from build123d import *

# Parameters (mm, degrees)
BOSS_EXTRUDE1_DEPTH = 20
BOSS_EXTRUDE2_DEPTH = 395
BOSS_EXTRUDE3_START = -30
BOSS_EXTRUDE3_DEPTH = 15
BOSS_EXTRUDE4_DEPTH = 5
BOSS_EXTRUDE5_DEPTH = 15
CHAMFER1_SIZE       = 10
BOSS_EXTRUDE8_DEPTH = 20
FILLET1_R           = 5
CHAMFER2_SIZE       = 10


with BuildPart() as part:
    # Sketch1 → Boss-Extrude1 (new body)
    with BuildSketch(Plane(origin=(0, 0, 0), x_dir=(1, 0, 0), z_dir=(0, 1, 0))):
        Polygon((280, 0), (280, -320), (0, -320), (0, -50), (135, -50), (135, 0), align=None)
    extrude(amount=BOSS_EXTRUDE1_DEPTH)

    # Sketch2 → Boss-Extrude2 (add)
    with BuildSketch(Plane(origin=(0, 20, 0), x_dir=(1, 0, 0), z_dir=(0, 1, 0))):
        with BuildLine():
            Line((36, -60), (204, -60))
            ThreePointArc((204, -60), (215.313708499, -64.686291501), (220, -76))
            Line((220, -76), (220, -244))
            ThreePointArc((220, -244), (215.313708499, -255.313708499), (204, -260))
            Line((204, -260), (36, -260))
            ThreePointArc((36, -260), (24.686291501, -255.313708499), (20, -244))
            Line((20, -244), (20, -76))
            ThreePointArc((20, -76), (24.686291501, -64.686291501), (36, -60))
        make_face()
        with BuildLine():
            Line((36, -68), (204, -68))
            ThreePointArc((204, -68), (209.656854249, -70.343145751), (212, -76))
            Line((212, -76), (212, -244))
            ThreePointArc((212, -244), (209.656854249, -249.656854249), (204, -252))
            Line((204, -252), (36, -252))
            ThreePointArc((36, -252), (30.343145751, -249.656854249), (28, -244))
            Line((28, -244), (28, -76))
            ThreePointArc((28, -76), (30.343145751, -70.343145751), (36, -68))
        make_face(mode=Mode.SUBTRACT)
    extrude(amount=BOSS_EXTRUDE2_DEPTH)

    # Sketch3 → Boss-Extrude3 (add)
    with BuildSketch(Plane.XY.offset(260).offset(BOSS_EXTRUDE3_START)):
        Polygon((230, 20), (270, 20), (270, 50), (250, 320), (220, 320), (220, 30), align=None)
    boss_extrude3 = extrude(amount=-BOSS_EXTRUDE3_DEPTH)

    # Mirror1: Boss-Extrude3 across plane
    add(boss_extrude3.mirror(Plane(origin=(0, 0, 160), x_dir=(1, 0, 0), z_dir=(0, 0, -1))))

    # Sketch4 → Boss-Extrude4 (add)
    with BuildSketch(Plane(origin=(0, 415, 0), x_dir=(1, 0, 0), z_dir=(0, 1, 0))):
        Polygon((30, -65), (210, -65), (215, -70), (215, -250), (210, -255), (30, -255), (25, -250), (25, -70), align=None)
    extrude(amount=BOSS_EXTRUDE4_DEPTH)

    # Sketch5 → Boss-Extrude5 (add)
    with BuildSketch(Plane.ZY.offset(-20)):
        Polygon((90, 405), (230, 405), (240, 395), (240, 255), (230, 245), (90, 245), (80, 255), (80, 395), align=None)
    extrude(amount=BOSS_EXTRUDE5_DEPTH)

    # Chamfer1
    chamfer1_edges = [part.edges().sort_by_distance(p)[0] for p in [
        (280, 10, 0),
        (280, 10, 320),
        (0, 10, 320),
        (0, 10, 50),
    ]]
    chamfer(chamfer1_edges, length=CHAMFER1_SIZE)

    # Sketch8 → Boss-Extrude8 (add)
    with BuildSketch(Plane(origin=(0, 0, 60), x_dir=(-1, 0, 0), z_dir=(0, 0, -1))):
        Polygon((-118, 399), (-53, 399), (-43, 389), (-43, 59), (-53, 49), (-118, 49), (-128, 59), (-128, 389), align=None)
    extrude(amount=BOSS_EXTRUDE8_DEPTH)

    # Fillet1
    fillet1_edges = [part.edges().sort_by_distance(p)[0] for p in [
        (135, 10, 50),
    ]]
    fillet(fillet1_edges, radius=FILLET1_R)

    # Chamfer2
    chamfer2_edges = [part.edges().sort_by_distance(p)[0] for p in [
        (135, 10, 0),
    ]]
    chamfer(chamfer2_edges, length=CHAMFER2_SIZE)


solid = part.part
Can you work these out from the model? Positions are in its coordinate system, mm. A direction names the side the tool comes from. Coordinates: 2 decimals unless noted, no trailing zeros. Write each loop counter-clockwise with the first axis right and the second up, starting at its lowest first coordinate (ties: lowest second). Pieces come first, ordered by that corner, then holes.
Q1. If we mould it in two halves opening along X, with no side actions, what happens to faces 1 (the face through (48, 54, 50)), 2 (the face through (121, 20, 159)), 3 (the face through (13, 405, 159)), 4 (the face through (212, 215, 159))? For each: +X half, -X half, draft (parallel to the pull), parting line (faces both ways), or undercut.
Results found:
face 1: -X half
face 2: undercut
face 3: draft
face 4: undercut
Q2. Imagine slicing it at D-D, the plane y = 381. List the corners of the cut face in (x, z) for me, plus the area to 3 significant figures.
Results found:
outline: (5, 80) - (20, 80) - (20, 76) arc R16 ccw to (36, 60) - (43, 60) - (43, 40) - (128, 40) - (128, 60) - (204, 60) arc R16 ccw to (220, 76) - (220, 244) arc R16 ccw to (204, 260) - (36, 260) arc R16 ccw to (20, 244) - (20, 240) - (5, 240) - close; hole (28, 76) arc R8 ccw to (36, 68) - (204, 68) arc R8 ccw to (212, 76) - (212, 244) arc R8 ccw to (204, 252) - (36, 252) arc R8 ccw to (28, 244) - close
area: 10,100 mm2
Q3. Imagine slicing it at A-A, the plane y = 117.5. List the corners of the cut face in (x, z) for me, plus the area to 3 significant figures.
Results found:
outline: (20, 76) arc R16 ccw to (36, 60) - (43, 60) - (43, 40) - (128, 40) - (128, 60) - (204, 60) arc R16 ccw to (220, 76) - (220, 90) - (265, 90) - (265, 105) - (220, 105) - (220, 215) - (265, 215) - (265, 230) - (220, 230) - (220, 244) arc R16 ccw to (204, 260) - (36, 260) arc R16 ccw to (20, 244) - close; hole (28, 76) arc R8 ccw to (36, 68) - (204, 68) arc R8 ccw to (212, 76) - (212, 244) arc R8 ccw to (204, 252) - (36, 252) arc R8 ccw to (28, 244) - close
area: 9,030 mm2
Q4. Imagine slicing it at B-B, the plane x = 82.5. List the corners of the cut face in (y, z) for me.
Results found:
outline: (0, 50) - (20, 50) - (20, 60) - (49, 60) - (49, 40) - (399, 40) - (399, 60) - (415, 60) - (415, 65) - (420, 65) - (420, 255) - (415, 255) - (415, 260) - (20, 260) - (20, 320) - (0, 320) - close; hole (20, 68) - (415, 68) - (415, 252) - (20, 252) - close
Q5. Which directions (+Z, -Z, +X, -X, +Y, -Y) give clear straight access to the entire face, cutting with the end or side of a thin tool? Please do faces 5 (the face through (69, 10, 50)), 6 (the face through (24.563, 214.735, 64.811)), 7 (the face through (235, 320, 97)), 8 (the face through (86, 399, 50)).
Results found:
face 5: -Z, -X, -Y
face 6: -Z, -X, +Y
face 7: +Z, -Z, +X, +Y
face 8: -Z, +X, -X, +Y
Q6. For P1, Ø4, axis at x = 226, y = 121.5, coming from the -Z side; P2, Ø2, axis at x = 57, y = 113, coming from the -Z side; P3, Ø16.5, axis at x = 14.5, z = 141, coming from the +Y side, each with a flat end and sliding along its axis, tell me the tip position at first contact or that it passes through.
Results found:
P1: stops at z = 90
P2: stops at z = 40
P3: stops at y = 415
Q7. Imagine slicing it at C-C, the plane x = 235. List the corners of the cut face in (y, z) for me.
Results found:
outline: (0, 0) - (20, 0) - (20, 90) - (320, 90) - (320, 105) - (20, 105) - (20, 215) - (320, 215) - (320, 230) - (20, 230) - (20, 320) - (0, 320) - close
Q8. Please list where these lines run through material, in increasing order: L1, parallel to X at y = 172, z = 145; L2, parallel to Y at x = 167.5, z = 224.5; L3, parallel to X at y = 247.5, z = 117.5.
Results found:
L1: x = 20 to 28, 212 to 220
L2: y = 0 to 20, 415 to 420
L3: x = 5 to 28, 212 to 220
